```python
from build123d import *

# Parameters (mm, degrees)
SKETCH_1_W          = 55
SKETCH_1_H          = 35
SKETCH_1_R          = 11.5
EXTRUDE_1_DEPTH     = 2
CUT_EXTRUDE_1_REACH = 34.841
SKETCH_2_R          = 3
CHAMFER_1_SIZE      = 2


with BuildPart() as part:
    # Sketch 1 → Extrude 1 (new, symmetric)
    with BuildSketch(Plane.XY):
        Rectangle(SKETCH_1_W, SKETCH_1_H)
        Circle(SKETCH_1_R, mode=Mode.SUBTRACT)
    extrude(amount=EXTRUDE_1_DEPTH, both=True)

    # Sketch 2 → Cut-Extrude 1 (cut, up to next)
    with BuildSketch(Plane.XY.offset(2), mode=Mode.PRIVATE) as cut_extrude_1_sk1:
        with Locations((-21.5, 11.5)):
            Circle(SKETCH_2_R)
    cut_extrude_1_tool1 = extrude(cut_extrude_1_sk1.sketch, amount=-CUT_EXTRUDE_1_REACH, mode=Mode.PRIVATE) & part.part
    # Sketch 2 → Cut-Extrude 1 (cut, up to next)
    with BuildSketch(Plane.XY.offset(2), mode=Mode.PRIVATE) as cut_extrude_1_sk2:
        with Locations((21.5, 11.5)):
            Circle(SKETCH_2_R)
    cut_extrude_1_tool2 = extrude(cut_extrude_1_sk2.sketch, amount=-CUT_EXTRUDE_1_REACH, mode=Mode.PRIVATE) & part.part
    cut_extrude_1_1 = cut_extrude_1_tool1.solids().sort_by_distance((-21.5, 11.5, 2))[0]
    add(cut_extrude_1_1, mode=Mode.SUBTRACT)
    cut_extrude_1_2 = cut_extrude_1_tool2.solids().sort_by_distance((21.5, 11.5, 2))[0]
    add(cut_extrude_1_2, mode=Mode.SUBTRACT)
    cut_extrude_1 = cut_extrude_1_1 + cut_extrude_1_2  # Cut-Extrude 1 as one shape, for the pattern or mirror that repeats it

    # Chamfer 1
    chamfer_1_edges = [part.edges().sort_by_distance(p)[0] for p in [
        (27.5, -17.5, 0),
        (-27.5, -17.5, 0),
        (-27.5, 17.5, 0),
        (27.5, 17.5, 0),
    ]]
    chamfer(chamfer_1_edges, length=CHAMFER_1_SIZE)

    # Mirror 1: Cut-Extrude 1 across plane
    add(cut_extrude_1.mirror(Plane.ZX), mode=Mode.SUBTRACT)


solid = part.part
```
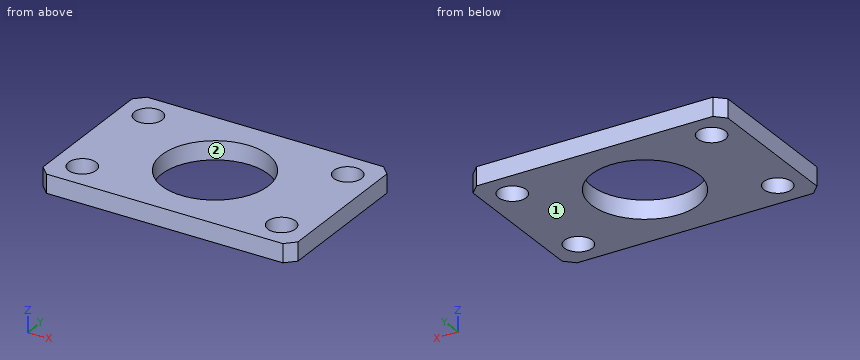
Design review of the part built by this model. Coordinates are the model's own, in mm. Face numbers are marked on the shaded views. Round coordinates to 2 decimals unless told otherwise and drop trailing zeros. Order: outer loops, then holes, each group sorted by start corner. A loop starts at its lowest first (then second) coordinate and runs counter-clockwise, first axis right, second up. Notation, with made-up numbers: (57, 64.5) - (71, 64.5) arc R36 cw to (71, 103.5) - close; hole circle Ø6 at (73, -22). An arc over 180 degrees is marked (long way). Return JSON: item names as keys, results as strings.
Q1. Consider section D-D on x = 0. Write out the cut boundary in (y, z).
Computed values:
{"outline": "(-17.5, -2) - (-11.5, -2) - (-11.5, 2) - (-17.5, 2) - close; (11.5, -2) - (17.5, -2) - (17.5, 2) - (11.5, 2) - close"}
Q2. The part is to be moulded in two halves that separate along X. For the marked faces 1 and 2, say which applies: pulls with the +X half, pulls with the -X half, needs draft (parallel to the pull), parting line crosses it, or undercut.
Computed values:
{"face 1": "needs draft", "face 2": "undercut"}
Q3. Consider section B-B on z = -0.5. Write out the cut boundary in (x, y).
Computed values:
{"outline": "(-27.5, -15.5) - (-25.5, -17.5) - (25.5, -17.5) - (27.5, -15.5) - (27.5, 15.5) - (25.5, 17.5) - (-25.5, 17.5) - (-27.5, 15.5) - close; hole circle Ø6 at (-21.5, -11.5); hole circle Ø6 at (-21.5, 11.5); hole circle Ø23 at (0, 0); hole circle Ø6 at (21.5, -11.5); hole circle Ø6 at (21.5, 11.5)"}
Q4. Consider section A-A on x = -21.5. Write out the cut boundary in (y, z).
Computed values:
{"outline": "(-17.5, -2) - (-14.5, -2) - (-14.5, 2) - (-17.5, 2) - close; (-8.5, -2) - (8.5, -2) - (8.5, 2) - (-8.5, 2) - close; (14.5, -2) - (17.5, -2) - (17.5, 2) - (14.5, 2) - close"}
Q5. Consider section C-C on y = 0. Write out the cut boundary in (x, z), plus the area to 3 significant figures.
Computed values:
{"outline": "(-27.5, -2) - (-11.5, -2) - (-11.5, 2) - (-27.5, 2) - close; (11.5, -2) - (27.5, -2) - (27.5, 2) - (11.5, 2) - close", "area": "128 mm2"}
Q6. Wall thickness on L1, parallel to Y at x = -21.5, z = 1.05; L2, parallel to Y at x = 0, z = 1.1; L3, parallel to Y at x = -5, z = 0.1: over which ranges is each line inside the solid? List them lowest first. Write a range as [from, to].
Computed values:
{"L1": "y = [-17.5, -14.5], [-8.5, 8.5], [14.5, 17.5]", "L2": "y = [-17.5, -11.5], [11.5, 17.5]", "L3": "y = [-17.5, -10.36], [10.36, 17.5]"}
